```python
from build123d import *

# Parameters (mm, degrees)
SKETCH_1_R               = 6
SKETCH_1_R_2             = 5.5
EXTRUDE_1_DEPTH          = 246.5
CUT_EXTRUDE_1_DEPTH      = 247.646001387
CUT_EXTRUDE_1_DEPTH_BACK = 247.646001387
SKETCH_2_R               = 1.55


with BuildPart() as part:
    # 草图1 → 凸台-拉伸1 (new body)
    with BuildSketch(Plane(origin=(0, 0, 0), x_dir=(1, 0, 0), z_dir=(0, 1, 0))):
        with Locations(Location((0, 0, 0), (0, 0, 270))):
            Circle(SKETCH_1_R)
        with Locations(Location((0, 0, 0), (0, 0, 270))):
            Circle(SKETCH_1_R_2, mode=Mode.SUBTRACT)
    extrude(amount=EXTRUDE_1_DEPTH)

    # 草图2 → 切除-拉伸1 (cut, two sides: drawn at the far end of the back side and taken through both)
    with BuildSketch(Plane.XY.offset(-CUT_EXTRUDE_1_DEPTH_BACK)):
        with Locations((0, 237)):
            Circle(SKETCH_2_R)
        with Locations((0, 9.5)):
            Circle(SKETCH_2_R)
    extrude(amount=CUT_EXTRUDE_1_DEPTH + CUT_EXTRUDE_1_DEPTH_BACK, mode=Mode.SUBTRACT)


solid = part.part
```
Source: CAD feature listing. Evaluate the final solid. Frame: model axes, mm. Coordinates: 2 decimals unless noted, no trailing zeros. Loops run counter-clockwise (first coordinate to the right, second up) from the corner with the lowest first, then second, coordinate; pieces in that order, holes last. Notation, with made-up numbers: M 21,-28.75 L 79,-28.75 A5 cw 79,-19.75 Z; hole C 24,69 d6. An arc over 180 degrees is marked long. Put each result on its own line as item: value. Start each with the question number.
1) Cut plane A-A on z = 0. Return the cut outline in (x, y), then the cut area to 4 significant figures.
2) Pull-direction query (X, two-part tool) for faces 1 (the face through (1.802, 121.524, 5.723)), 2 (the face through (-5, 0, 3)), 3 (the face through (-5.37, 121.52, -1.19)); classes: pulls with the +X half, pulls with the -X half, needs draft (parallel to the pull), parting line crosses it, or undercut.
3) Cut plane B-B on y = 226.5. Return the cut outline in (x, z), then the cut area to 3 significant figures.
4) Ray query, L1, parallel to Y at x = 0, z = 5.95; L2, parallel to Z at x = 1, y = 89.5; L3, parallel to X at y = 9.5, z = 5.5. Return the intervals inside material, ascending. Write a range as from..to.
5) Contact query for flat-ended pins moving along their axis: pin 1 Ø5 at (x, z) = (-4.5, -3.5) entering from -Y; pin 2 Ø6 at (y, z) = (58.5, -4) entering from -X; pin 3 Ø1 at (x, z) = (-2, 4) entering from -Y. Output: stop coordinate, or through.
The answers:
1. outline: M -6,0 L -5.5,0 L -5.5,246.5 L -6,246.5 Z; M 5.5,0 L 6,0 L 6,246.5 L 5.5,246.5 Z
1. area: 246.5 mm²
2. face 1: parting line crosses it
2. face 2: needs draft
2. face 3: undercut
3. outline: C 0,0 d12; hole C 0,0 d11
3. area: 18.1 mm²
4. L1: y = 0..7.95, 11.05..235.45, 238.55..246.5
4. L2: z = -5.92..-5.41, 5.41..5.92
4. L3: x = -2.4..-1.55, 1.55..2.4
5. pin 1: stops at y = 0
5. pin 2: stops at x = -5.92
5. pin 3: passes through
